Input: part model. Units: mm. Frame: model coordinates. A direction names the side the tool comes from. Round coordinates to 2 decimals unless told otherwise and drop trailing zeros. Loops run counter-clockwise (first coordinate to the right, second up) from the corner with the lowest first, then second, coordinate; pieces in that order, holes last.
(1) Access query for faces 4 (the face through (-0.715, -32.492, 26.768)), 5 (the face through (-45.292, -21.801, 12.648)), 6 (the face through (0.715, -32.492, 1.268)), 7 (the face through (0, -32, 12)), 8 (the face through (1, -36, 0)). Directions: +Z, -Z, +X, -X, +Y, -Y. A direction counts if a zero-diameter tool reaches every point of the face in a straight line with its end or side. Return the directions, or none.
(2) Cut plane D-D, the plane z = 8.25. Output: boundary loops of the cut face in (x, y).
(3) Line query: line 1 (X direction, y = -17, z = 13); line 2 (Z direction, x = -41, y = -24); line 3 (Y direction, x = -0.5, z = 11). Output: solid intervals per line, ascending.
(4) First-contact query: pin 1 Ø3 at (x, z) = (-15.5, 17.5) entering from +Y; pin 2 Ø10 at (x, y) = (-13, -23.5) entering from -Z; pin 3 Ø1.2 at (x, z) = (0, 13) entering from +Y. Flat tips, straight axial feed; report the tip coordinate or a pass-through.
(5) Cut plane A-A, the plane x = -41. Output: boundary loops of the cut face in (y, z), and give its area (3 significant figures).
(6) Cut plane C-C, the plane y = -31.5. Output: boundary loops of the cut face in (x, z), and give its area (3 significant figures).
(7) Draft query along X for faces 1 (the face through (0, -34, 14)), 2 (the face through (-36, 0, 14)), 3 (the face through (50, -21, 14)). Return one class per face: released by +X, released by -X, zero draft, split by the parting line, or undercut.
(8) Cut plane B-B, the plane z = 14. Output: boundary loops of the cut face in (x, y), and give its area (3 significant figures).
from build123d import *

# Parameters (mm, degrees)
BOSS_EXTRUDE1_DEPTH = 28
SKETCH2_R           = 32.5
CUT_EXTRUDE1_DEPTH  = 2.5
CUT_EXTRUDE2_START  = -2.5
SKETCH3_R           = 32.5
CUT_EXTRUDE2_DEPTH  = 2.5
CHAMFER1_SIZE       = 0.3
HOLE1_D             = 9
HOLE2_D             = 4
HOLE2_DEPTH         = 34


with BuildPart() as part:
    # Sketch1 → Boss-Extrude1 (new body)
    with BuildSketch(Plane.XY):
        with BuildLine():
            Line((-50, 0), (-30, 0))
            ThreePointArc((-30, 0), (0, -30), (30, 0))
            Line((30, 0), (50, 0))
            Line((50, 0), (50, -43))
            Line((50, -43), (-50, -43))
            Line((-50, -43), (-50, 0))
        make_face()
    extrude(amount=BOSS_EXTRUDE1_DEPTH)

    # Sketch2 → Cut-Extrude1 (cut)
    with BuildSketch(Plane.XY.offset(28)):
        Circle(SKETCH2_R)
    extrude(amount=-CUT_EXTRUDE1_DEPTH, mode=Mode.SUBTRACT)

    # Sketch3 → Cut-Extrude2 (cut)
    with BuildSketch(Plane(origin=(0, 0, 0), x_dir=(-1, 0, 0), z_dir=(0, 0, -1)).offset(CUT_EXTRUDE2_START)):
        Circle(SKETCH3_R)
    extrude(amount=CUT_EXTRUDE2_DEPTH, mode=Mode.SUBTRACT)

    # Chamfer1
    chamfer1_edges = [part.edges().sort_by_distance(p)[0] for p in [
        (0, -30, 25.5),
        (0, -30, 2.5),
    ]]
    chamfer(chamfer1_edges, length=CHAMFER1_SIZE)

    # Hole1 (through all)
    with Locations(Plane(origin=(0, 0, 0), x_dir=(1, 0, 0), z_dir=(0, 1, 0))):
        with Locations((-41, -14), (41, -14)):
            Hole(HOLE1_D / 2)

    # Hole2
    with Locations(Plane(origin=(0, 0, 0), x_dir=(1, 0, 0), z_dir=(0, 1, 0))):
        with Locations((0, -14)):
            Hole(HOLE2_D / 2, depth=HOLE2_DEPTH)


solid = part.part
Reported:
1. face 4: +Z, +Y
1. face 5: +Y, -Y
1. face 6: -Z, +Y
1. face 7: +Y
1. face 8: -Z, +X, -X, +Y, -Y
2. outline: (-50, -43) - (50, -43) - (50, 0) - (30, 0) arc R30 cw to (-30, 0) - (-50, 0) - close
3. line 1: x = -50 to -45.39, -36.61 to -24.72, 24.72 to 36.61, 45.39 to 50
3. line 2: z = 0 to 9.5, 18.5 to 28
3. line 3: y = -43 to -30
4. pin 1: stops at y = -24.72
4. pin 2: stops at z = 2.5
4. pin 3: stops at y = -34
5. outline: (-43, 0) - (0, 0) - (0, 9.5) - (-43, 9.5) - close; (-43, 18.5) - (0, 18.5) - (0, 28) - (-43, 28) - close
5. area: 817 mm2
6. outline: (-50, 0) - (-8, 0) - (-8, 2.5) - (8, 2.5) - (8, 0) - (50, 0) - (50, 28) - (8, 28) - (8, 25.5) - (-8, 25.5) - (-8, 28) - (-50, 28) - close; hole circle Ø9 at (-41, 14); hole circle Ø4 at (0, 14); hole circle Ø9 at (41, 14)
6. area: 2,580 mm2
7. face 1: undercut
7. face 2: zero draft
7. face 3: released by +X
8. outline: (-50, -43) - (-45.5, -43) - (-45.5, 0) - (-50, 0) - close; (-36.5, -43) - (36.5, -43) - (36.5, 0) - (30, 0) arc R30 cw to (2, -29.93) - (2, -34) - (-2, -34) - (-2, -29.93) arc R30 cw to (-30, 0) - (-36.5, 0) - close; (45.5, -43) - (50, -43) - (50, 0) - (45.5, 0) - close
8. area: 2,100 mm2
